Read the model definition and answer for the solid it produces. Units are mm, in the model's axes. Coordinates: 2 decimals unless noted, no trailing zeros. Write each loop counter-clockwise with the first axis right and the second up, starting at its lowest first coordinate (ties: lowest second). Pieces come first, ordered by that corner, then holes.
(1) Straight lines are drawn through the part: line 1 along X through (y, z) = (1.25, 87); line 2 along X through (y, z) = (2.5, 83); line 3 along Z through (x, y) = (56.5, 3.5). For each, find the intervals that lie inside material, in ascending order.
(2) The part is cut by section A-A, the plane y = 1.5. Determine the outline of the cut face in (x, z), and give its area (3 significant figures).
(3) Given pin 1 (6.5 mm diameter, centred on x = 58.737, z = 84.137, fed in from -Y); pin 2 (5 mm diameter, centred on x = -37, z = -39, fed in from -Y), each flat-ended and moving along its own axis, determine where each tip first touches the part or whether it passes through.
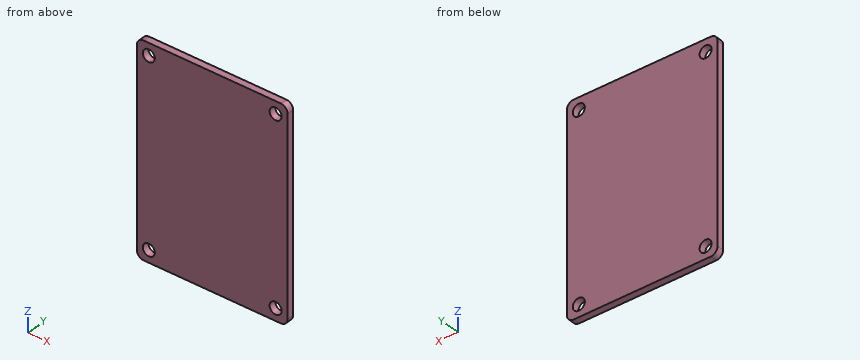
```python
from build123d import *

# Parameters (mm, degrees)
SKETCH1_W                      = 139.7
SKETCH1_H                      = 190.5
BOSS_EXTRUDE1_DEPTH            = 6.35
FILLET1_R                      = 6.35
F_7_16_0_4375_DIAMETER_HOLE1_D = 11.1125
LPATTERN1_COUNT                = 2
LPATTERN1_PITCH                = 168.275
LPATTERN1_COUNT_DIR2           = 2
LPATTERN1_PITCH_DIR2           = 117.475


with BuildPart() as part:
    # Sketch1 → Boss-Extrude1 (new body)
    with BuildSketch(Plane(origin=(0, 0, 0), x_dir=(1, 0, 0), z_dir=(0, 1, 0))):
        Rectangle(SKETCH1_W, SKETCH1_H)
    extrude(amount=BOSS_EXTRUDE1_DEPTH)

    # Fillet1
    fillet1_edges = [part.edges().sort_by_distance(p)[0] for p in [
        (-69.85, 3.175, -95.25),
        (69.85, 3.175, -95.25),
        (69.85, 3.175, 95.25),
        (-69.85, 3.175, 95.25),
    ]]
    fillet(fillet1_edges, radius=FILLET1_R)

    # 7/16 (0.4375) Diameter Hole1 (through all)
    with Locations(Plane(origin=(0, 6.35, 0), x_dir=(1, 0, 0), z_dir=(0, 1, 0))):
        with Locations((-58.738, 84.138)):
            f_7_16_0_4375_diameter_hole1 = Hole(F_7_16_0_4375_DIAMETER_HOLE1_D / 2)

    # LPattern1: 7_16 _0.4375_ Diameter Hole1 2 × 2
    with Locations(*[(j * LPATTERN1_PITCH_DIR2, 0, i * LPATTERN1_PITCH) for i in range(LPATTERN1_COUNT) for j in range(LPATTERN1_COUNT_DIR2) if (i, j) != (0, 0)]):
        add(f_7_16_0_4375_diameter_hole1, mode=Mode.SUBTRACT)


solid = part.part
```
Computed:
1. line 1: x = -69.85 to -63.5, -53.98 to 53.98, 63.5 to 69.85
1. line 2: x = -69.85 to -64.18, -53.3 to 53.3, 64.18 to 69.85
1. line 3: z = -95.25 to -89.22, -79.05 to 79.05, 89.22 to 95.25
2. outline: (-69.85, -88.9) arc R6.35 ccw to (-63.5, -95.25) - (63.5, -95.25) arc R6.35 ccw to (69.85, -88.9) - (69.85, 88.9) arc R6.35 ccw to (63.5, 95.25) - (-63.5, 95.25) arc R6.35 ccw to (-69.85, 88.9) - close; hole circle Ø11.11 at (-58.74, -84.14); hole circle Ø11.11 at (-58.74, 84.14); hole circle Ø11.11 at (58.74, -84.14); hole circle Ø11.11 at (58.74, 84.14)
2. area: 26,200 mm2
3. pin 1: passes through
3. pin 2: stops at y = 0
